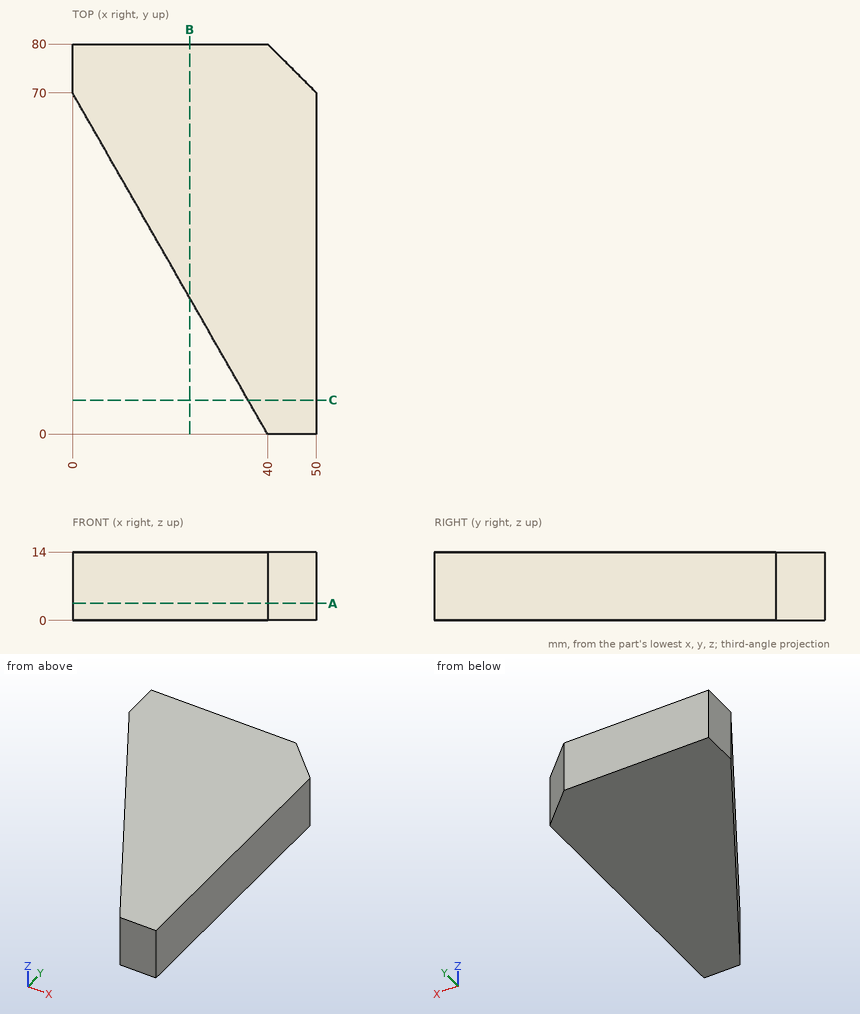
The drawing under review shows one solid part. Ordinate dimensions are in mm from its lowest x, y, z. Round coordinates to 2 decimals unless told otherwise and drop trailing zeros. Write each loop counter-clockwise with the first axis right and the second up, starting at its lowest first coordinate (ties: lowest second). Pieces come first, ordered by that corner, then holes. Notation, with made-up numbers: (45.5, -8.5) - (85.5, -8.5) arc R10 cw to (85.5, 2.5) - close; hole circle Ø8 at (-3.5, -27.5). An arc over 180 degrees is marked (long way). Use a Markdown table: item, result. Add a question column.
1. Wall thickness on probe 1 along Y at (x, z) = (32, 7.5); probe 2 along X at (y, z) = (30.5, 5.25); probe 3 along Y at (x, z) = (28.5, 1) (3 decimals): over which ranges is each line inside the solid? List them lowest first.
2. We need section B-B (x = 24). State the section outline as (y, z) points, then the cut area to 3 significant figures.
3. We need section C-C (y = 7). State the section outline as (x, z) points.
4. We need section A-A (z = 3.5). State the section outline as (x, y) points.
5. Clearance check with flat-ended pins moving along their axes: pin 1 (1.5 mm diameter, centred on y = 35.5, z = 11, fed in from -X); pin 2 (12 mm diameter, centred on x = 36, y = 71.5, fed in from -Z); pin 3 (8 mm diameter, centred on x = 44.5, z = 11, fed in from +Y); pin 4 (3 mm diameter, centred on x = 27.5, z = 11, fed in from -Y). State where each tip first meets the part, or that it passes through.
Output:
| question | item | result |
|---|---|---|
| 1 | probe 1 | y = 14 to 80 |
| 1 | probe 2 | x = 22.57 to 50 |
| 1 | probe 3 | y = 20.125 to 80 |
| 2 | outline | (28, 0) - (80, 0) - (80, 14) - (28, 14) - close |
| 2 | area | 728 mm2 |
| 3 | outline | (36, 0) - (50, 0) - (50, 14) - (36, 14) - close |
| 4 | outline | (0, 70) - (40, 0) - (50, 0) - (50, 70) - (40, 80) - (0, 80) - close |
| 5 | pin 1 | stops at x = 19.29 |
| 5 | pin 2 | stops at z = 0 |
| 5 | pin 3 | stops at y = 79.5 |
| 5 | pin 4 | stops at y = 19.25 |
